```python
from build123d import *

# Parameters (mm, degrees)
EXTRUDE_1_DEPTH     = 20
CUT_EXTRUDE_1_DEPTH = 162.052786378


with BuildPart() as part:
    # 草图1 → 凸台-拉伸1 (new body)
    with BuildSketch(Plane.XY):
        with BuildLine():
            Line((45, 15), (113, 15))
            Line((113, 15), (113, 24.5))
            ThreePointArc((113, 24.5), (50.421049865, 50.421049865), (24.5, 113))
            Line((24.5, 113), (15, 113))
            Line((15, 113), (15, 45))
            ThreePointArc((15, 45), (10.606601718, 34.393398282), (0, 30))
            ThreePointArc((0, 30), (-10.606601718, 34.393398282), (-15, 45))
            Line((-15, 45), (-15, 113))
            Line((-15, 113), (-24.5, 113))
            ThreePointArc((-24.5, 113), (-50.421049865, 50.421049865), (-113, 24.5))
            Line((-113, 24.5), (-113, 15))
            Line((-113, 15), (-45, 15))
            ThreePointArc((-45, 15), (-34.393398282, 10.606601718), (-30, 0))
            ThreePointArc((-30, 0), (-34.393398282, -10.606601718), (-45, -15))
            Line((-45, -15), (-113, -15))
            Line((-113, -15), (-113, -24.5))
            ThreePointArc((-113, -24.5), (-50.421049865, -50.421049865), (-24.5, -113))
            Line((-24.5, -113), (-15, -113))
            Line((-15, -113), (-15, -45))
            ThreePointArc((-15, -45), (-10.606601718, -34.393398282), (0, -30))
            ThreePointArc((0, -30), (10.606601718, -34.393398282), (15, -45))
            Line((15, -45), (15, -113))
            Line((15, -113), (24.5, -113))
            ThreePointArc((24.5, -113), (50.421049865, -50.421049865), (113, -24.5))
            Line((113, -24.5), (113, -15))
            Line((113, -15), (45, -15))
            ThreePointArc((45, -15), (34.393398282, -10.606601718), (30, 0))
            ThreePointArc((30, 0), (34.393398282, 10.606601718), (45, 15))
        make_face()
    extrude(amount=EXTRUDE_1_DEPTH)

    # 草图2 → 切除-拉伸1 (cut, through all)
    with BuildSketch(Plane.XY.offset(20)):
        with BuildLine():
            Line((-4, 19), (4, 19))
            Line((4, 19), (4, 14.456832295))
            ThreePointArc((4, 14.456832295), (0, -15), (-4, 14.456832295))
            Line((-4, 14.456832295), (-4, 19))
        make_face()
    extrude(amount=-CUT_EXTRUDE_1_DEPTH, mode=Mode.SUBTRACT)


solid = part.part
```
The listing builds one solid part. Answer for the finished solid, in the listing's coordinates (mm). A direction names the side the tool comes from. Give positions to 0.01 mm unless a question says otherwise; leave off trailing zeros. Order: outer loops, then holes, each group sorted by start corner. A loop starts at its lowest first (then second) coordinate and runs counter-clockwise, first axis right, second up. Notation, with made-up numbers: (66, 44) - (88, 44) arc R13 cw to (88, 63) - close; hole circle Ø5 at (-24.75, -29.5). An arc over 180 degrees is marked (long way). Use one line per item in the form item = value. Start each with the question number.
(1) For faces 1 (the flat face through (-15, 79, 10)), 2 (the flat face through (15, -79, 10)), 3 (the flat face through (79, 15, 10)), 4 (the flat face through (-79, -15, 10)), determine the directions among +Z, -Z, +X, -X, +Y, -Y from which every point of the face is accessible in a straight line to the end or side of a thin tool.
(2) Consider line 1 (X direction, y = -70, z = 3.5); line 2 (Y direction, x = -100, z = 2); line 3 (X direction, y = -1.5, z = 17). Determine where each line is inside the solid, lowest interval first. Write a range as from..to.
(3) The mould has two halves that part along Y. Classify faces 5 (the flat face through (-79, 15, 10)), 6 (the cylindrical face through (-51.11, -49.74, 9.86)), 7 (the flat face through (20, 113, 10)): released by +Y, released by -Y, zero draft, split by the parting line, or undercut.
(4) A cutting plane is placed at C-C, the plane y = 73.5. Write down the section's boundary in (x, z), then the cut area to 3 significant figures.
(5) Flat-ended cylindrical pins translate along their axes: pin 1 Ø6 at (x, z) = (-70.5, 5) entering from -Y; pin 2 Ø2.5 at (x, z) = (-1, 10) entering from -Y; pin 3 Ø6 at (x, z) = (85.5, 8.5) entering from -Y. Find the tip coordinate at first contact, or state that the pin passes through.
(6) A cutting plane is placed at B-B, the plane x = -81. Write down the section's boundary in (y, z), then the cut area to 3 significant figures.
(7) A cutting plane is placed at A-A, the plane z = 17.25. Write down the section's boundary in (x, y), then the cut area to 3 significant figures.
Ans:
q1.face_1 = +Z, -Z, +Y
q1.face_2 = +Z, -Z, -Y
q1.face_3 = +Z, -Z, +X
q1.face_4 = +Z, -Z, -X
q2.line_1 = -35.65..-15, 15..35.65
q2.line_2 = -25.46..-15, 15..25.46
q2.line_3 = -30.08..-14.92, 14.92..30.08
q3.face_5 = undercut
q3.face_6 = released by -Y
q3.face_7 = released by +Y
q4.outline = (-33.8, 0) - (-15, 0) - (-15, 20) - (-33.8, 20) - close; (15, 0) - (33.8, 0) - (33.8, 20) - (15, 20) - close
q4.area = 752 mm^2
q5.pin_1 = -37.09
q5.pin_2 = -30.17
q5.pin_3 = -29.92
q6.outline = (-30.49, 0) - (-15, 0) - (-15, 20) - (-30.49, 20) - close; (15, 0) - (30.49, 0) - (30.49, 20) - (15, 20) - close
q6.area = 620 mm^2
q7.outline = (-113, -24.5) arc R88.5 cw to (-24.5, -113) - (-15, -113) - (-15, -45) arc R15 cw to (15, -45) - (15, -113) - (24.5, -113) arc R88.5 cw to (113, -24.5) - (113, -15) - (45, -15) arc R15 cw to (45, 15) - (113, 15) - (113, 24.5) arc R88.5 cw to (24.5, 113) - (15, 113) - (15, 45) arc R15 cw to (-15, 45) - (-15, 113) - (-24.5, 113) arc R88.5 cw to (-113, 24.5) - (-113, 15) - (-45, 15) arc R15 cw to (-45, -15) - (-113, -15) - close; hole (-4, 14.46) arc R15 ccw (long way) to (4, 14.46) - (4, 19) - (-4, 19) - close
q7.area = 16,200 mm^2
